Source: three-view drawing plus pictorial views. Frame: mm from the lowest corner of the part. A direction names the side the tool comes from. Coordinates: 2 decimals unless noted, no trailing zeros. Write each loop counter-clockwise with the first axis right and the second up, starting at its lowest first coordinate (ties: lowest second). Pieces come first, ordered by that corner, then holes. Notation, with made-up numbers: (54.5, 30) -> (78.5, 30) arc R29 ccw to (78.5, 68) -> close; hole circle Ø11 at (-29, 51). An arc over 180 degrees is marked (long way). Write item = value, one per line.
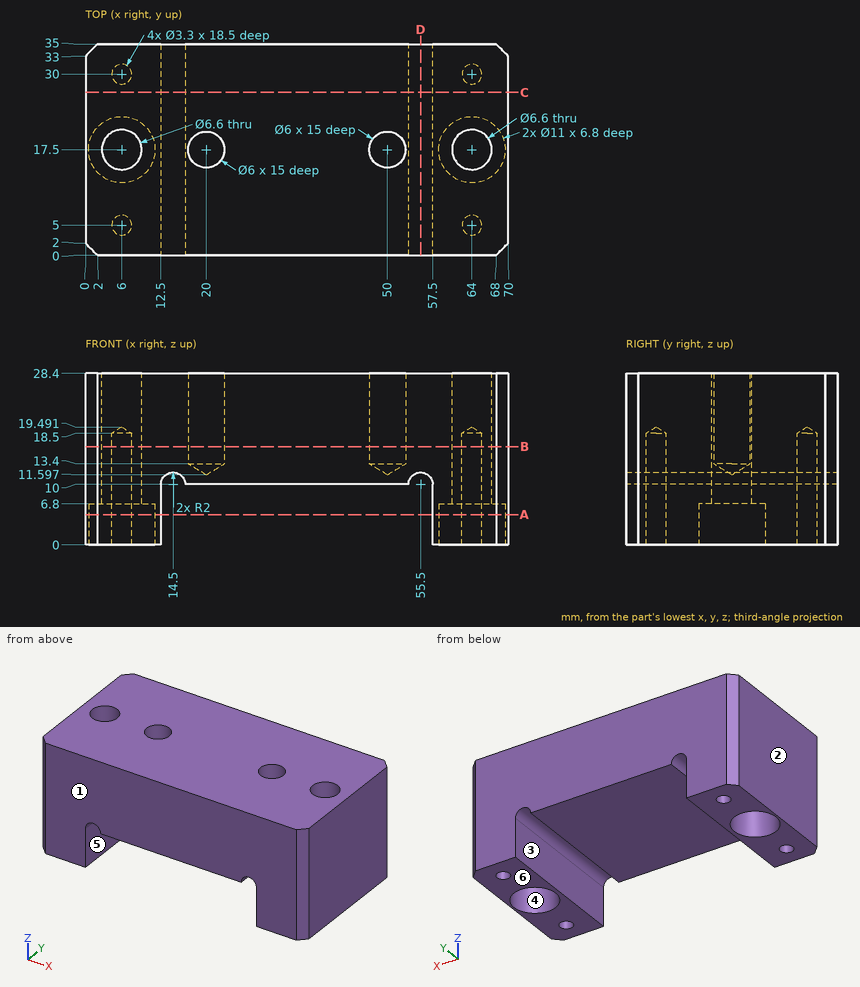
1) Cut plane A-A, the plane z = 5. Output: boundary loops of the cut face in (x, y).
Answer block:
outline = (0, 2) -> (2, 0) -> (12.5, 0) -> (12.5, 35) -> (2, 35) -> (0, 33) -> close; (57.5, 0) -> (68, 0) -> (70, 2) -> (70, 33) -> (68, 35) -> (57.5, 35) -> close; hole circle Ø11 at (6, 17.5); hole circle Ø3.3 at (6, 5); hole circle Ø3.3 at (6, 30); hole circle Ø11 at (64, 17.5); hole circle Ø3.3 at (64, 5); hole circle Ø3.3 at (64, 30)
2) First-contact query: pin 1 Ø5.5 at (x, y) = (64, 16) entering from -Z; pin 2 Ø2 at (x, y) = (6, 5) entering from -Z; pin 3 Ø3.5 at (x, y) = (5, 17) entering from -Z; pin 4 Ø8 at (x, y) = (28, 26.5) entering from -Z. Flat tips, straight axial feed; report the tip coordinate or a pass-through.
Answer block:
pin_1 = 6.8
pin_2 = 18.89
pin_3 = through
pin_4 = 10
3) Cut plane B-B, the plane z = 16.25. Give the number of separate pieces and of enclosed holes in the cut face, and give its area (3 significant figures).
Answer block:
separate_pieces = 1
enclosed_holes = 8
area = 2,280 mm2
4) Cut plane C-C, the plane y = 27. Output: boundary loops of the cut face in (x, z).
Answer block:
outline = (0, 0) -> (12.5, 0) -> (12.5, 10) arc R2 cw to (16.5, 10) -> (53.5, 10) arc R2 cw to (57.5, 10) -> (57.5, 0) -> (70, 0) -> (70, 28.4) -> (0, 28.4) -> close
5) Pull-direction query (X, two-part tool) for the marked faces 1, 2 and 3; classes: +X half, -X half, draft (parallel to the pull), parting line (faces both ways), or undercut.
Answer block:
face_1 = draft
face_2 = -X half
face_3 = undercut
6) Cut plane D-D, the plane x = 55.5. Output: boundary loops of the cut face in (y, z), and give its area (3 significant figures).
Answer block:
outline = (0, 12) -> (35, 12) -> (35, 28.4) -> (0, 28.4) -> close
area = 574 mm2
7) Material intervals for probe 1 along X at (y, z) = (30, 8.75); probe 2 along Y at (x, z) = (64, 14.75); probe 3 along Y at (x, z) = (50, 19), sorted ascending. Write a range as [from, to].
Answer block:
probe_1 = [0, 4.35], [7.65, 12.5], [57.5, 62.35], [65.65, 70]
probe_2 = [0, 3.35], [6.65, 14.2], [20.8, 28.35], [31.65, 35]
probe_3 = [0, 14.5], [20.5, 35]
8) Reachability of the marked faces 4, 5 and 6 from +Z, -Z, +X, -X, +Y, -Y: full face, straight path, thin tool, end or side. Return the list, or none.
Answer block:
face_4 = -Z
face_5 = -Z, +Y, -Y
face_6 = -Z, +X, -X, +Y, -Y
